from build123d import *

# Parameters (mm, degrees)
BOSS_EXTRUDE1_DEPTH = 158.75
SKETCH4_R           = 10.287
CUT_EXTRUDE1_DEPTH  = 184.15


with BuildPart() as part:
    # Sketch1 → Boss-Extrude1 (new, symmetric)
    with BuildSketch(Plane.XY):
        with BuildLine():
            Line((-10, 88.9), (0, 88.9))
            Line((0, 88.9), (0, -44.45))
            ThreePointArc((0, -44.45), (-7.735948816, -91.950507064), (-30.144264146, -134.541708966))
            Line((-30.144264146, -134.541708966), (-38.130619246, -128.523558734))
            ThreePointArc((-38.130619246, -128.523558734), (-17.219185368, -88.7774605), (-10, -44.45))
            Line((-10, -44.45), (-10, 88.9))
        make_face()
    extrude(amount=BOSS_EXTRUDE1_DEPTH, both=True)

    # Sketch4 → Cut-Extrude1 (cut, symmetric)
    with BuildSketch(Plane(origin=(0, 0, 0), x_dir=(0, 0, -1), z_dir=(1, 0, 0))):
        Circle(SKETCH4_R)
        with BuildLine():
            Line((-57.15, -101.6), (-57.15, -134.541708966))
            Line((-57.15, -134.541708966), (57.15, -134.541708966))
            Line((57.15, -134.541708966), (57.15, -101.6))
            ThreePointArc((57.15, -101.6), (0, -44.45), (-57.15, -101.6))
        make_face()
    extrude(amount=CUT_EXTRUDE1_DEPTH, both=True, mode=Mode.SUBTRACT)


solid = part.part
Geometry check sheet. Reference: the model listing, model coordinates, mm. A direction names the side the tool comes from. Give positions to 0.01 mm unless a question says otherwise; leave off trailing zeros. Order: outer loops, then holes, each group sorted by start corner. A loop starts at its lowest first (then second) coordinate and runs counter-clockwise, first axis right, second up. Notation, with made-up numbers: M -40,25.25 L 2,25.25 A35 ccw 2,60.25 Z; hole C 56.5,47 d11. An arc over 180 degrees is marked long. Use a Markdown table: item, result.
Item 1: Section check B-B (y = -116). Record the cut outline in (x, z).
Answers follow:
| item | result |
|---|---|
| outline | M -29.71,-158.75 L -18.21,-158.75 L -18.21,-57.15 L -29.71,-57.15 Z; M -29.71,57.15 L -18.21,57.15 L -18.21,158.75 L -29.71,158.75 Z |
Item 2: Draft check along Y on faces 1 (the flat face through (-34.082, -131.575, -107.239)), 2 (the cylindrical face through (-4.93, 10.2, 1.34)), 3 (the flat face through (0, 23, 2)). Enter one of: +Y half, -Y half, draft (parallel to the pull), parting line (faces both ways), or undercut.
Answers follow:
| item | result |
|---|---|
| face 1 | -Y half |
| face 2 | undercut |
| face 3 | draft |
Item 3: Section check C-C (z = -71.5). Record the cut outline in (x, y).
Answers follow:
| item | result |
|---|---|
| outline | M -38.13,-128.52 L -30.14,-134.54 A149.7 ccw 0,-44.45 L 0,88.9 L -10,88.9 L -10,-44.45 A139.7 cw Z |
Item 4: Section check A-A (y = 0). Record the cut outline in (x, z), and give its area (3 significant figures).
Answers follow:
| item | result |
|---|---|
| outline | M -10,-158.75 L 0,-158.75 L 0,-10.29 L -10,-10.29 Z; M -10,10.29 L 0,10.29 L 0,158.75 L -10,158.75 Z |
| area | 2,970 mm2 |
Item 5: Depth check by flat-ended pin: P1, Ø1.5, axis at y = -74.5, z = 80, coming from the -X side; P2, Ø10, axis at x = -11, z = -81, coming from the -Y side; P3, Ø1, axis at y = -51.5, z = 79, coming from the +X side. Enter the tip coordinate at first touch or a pass-through.
Answers follow:
| item | result |
|---|---|
| P1 | stops at x = -13.44 |
| P2 | stops at y = -111.79 |
| P3 | stops at x = -0.14 |
Item 6: Material ranges on line 1 along Y through (x, z) = (-6.25, 0); line 2 along X through (y, z) = (-19.5, 21.5); line 3 along X through (y, z) = (-56, 89), recorded low to high.
Answers follow:
| item | result |
|---|---|
| line 1 | y = -44.45 to -10.29, 10.29 to 88.9 |
| line 2 | x = -10 to 0 |
| line 3 | x = -10.48 to -0.45 |
Item 7: Section check D-D (y = 68.5). Record the cut outline in (x, z).
Answers follow:
| item | result |
|---|---|
| outline | M -10,-158.75 L 0,-158.75 L 0,158.75 L -10,158.75 Z |
Item 8: Tool access check on faces 4 (the flat face through (-5, 88.9, 2)), 5 (the flat face through (-10, 21, 2)), 6 (the flat face through (-25, -118, -57.15)). Record the directions out of +Z, -Z, +X, -X, +Y, -Y that give a thin tool (end or side, any length) a straight path to the whole face; none if there is none.
Answers follow:
| item | result |
|---|---|
| face 4 | +Z, -Z, +X, -X, +Y |
| face 5 | +Z, -Z, -X, +Y |
| face 6 | +X, -X, -Y |
